Here's how the part is built. I have some questions about the finished solid (model axes, mm). Face numbers are marked on the shaded views. A direction names the side the tool comes from. Give positions to 0.01 mm unless a question says otherwise; leave off trailing zeros. Write each loop counter-clockwise with the first axis right and the second up, starting at its lowest first coordinate (ties: lowest second). Pieces come first, ordered by that corner, then holes. Notation, with made-up numbers: (37, 69.5) - (46, 69.5) arc R35 cw to (46, 108.5) - close; hole circle Ø8 at (62, -12). An arc over 180 degrees is marked (long way). One line per item, written item: value. Start each with the question number.
1) Please list where these lines run through material, in increasing order: L1, parallel to X at y = -164, z = 3.75; L2, parallel to Z at x = 255.5, y = -168.75; L3, parallel to Y at x = 255, z = 1.5. Write a range as [from, to].
2) Imagine slicing it at C-C on x = 252.75. Write out the boundary of the cut face in (y, z).
3) Imagine slicing it at B-B on x = 257.25. Write out the boundary of the cut face in (y, z), plus the area to 3 significant figures.
4) Imagine slicing it at A-A on z = 0. Write out the boundary of the cut face in (x, y), plus the area to 3 significant figures.
5) I'm going to push flat-ended pins straight in: P1, Ø5, axis at x = 256.5, y = -165.5, coming from the +Z side; P2, Ø8, axis at x = 251, z = -0.5, coming from the +Y side; P3, Ø2, axis at x = 256.5, z = -4.5, coming from the -Y side. Where does each tip first touch, or does it pass through?
6) On a 3-axis mill with a long thin cutter (end or side, diameter ignored), from which of +Z, -Z, +X, -X, +Y, -Y can I reach the whole of each face in a straight line? I mean the marked faces 1 and 2. Say none if no direction works.
from build123d import *

# Parameters (mm, degrees)
CHAMFER_1_SIZE = 1


with BuildPart() as part:
    # 草图1 → 旋转1 (revolve)
    with BuildSketch(Plane.XY, mode=Mode.PRIVATE) as revolve_1_sk:
        Polygon((236.937142185, -170.509032878), (236.937142185, -164.259032878), (256.937142185, -164.259032878), (256.937142185, -160.509032878), (261.937142185, -160.509032878), (261.937142185, -170.509032878), align=None)
    revolve(revolve_1_sk.sketch.rotate(Axis((232.937142185, -170.509032878, 0), (1, 0, 0)), 90), axis=Axis((232.937142185, -170.509032878, 0), (1, 0, 0)))

    # 倒角1
    chamfer_1_edges = [part.edges().sort_by_distance(p)[0] for p in [
        (261.937142185, -170.509032878, -10),
        (256.937142185, -170.509032878, -10),
        (236.937142185, -170.509032878, -6.25),
    ]]
    chamfer(chamfer_1_edges, length=CHAMFER_1_SIZE)


solid = part.part
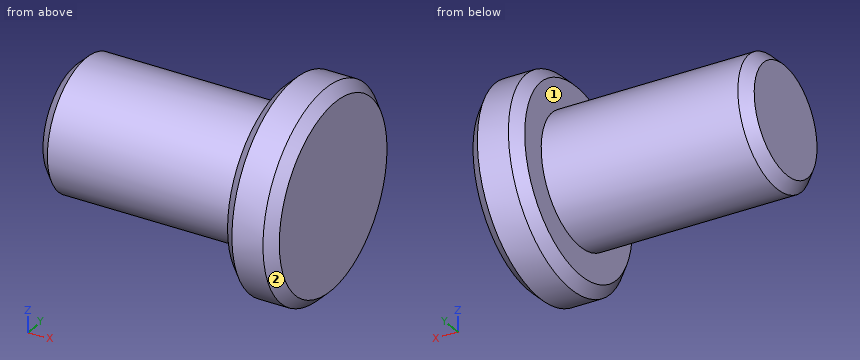
Numbers:
1. L1: [256.94, 261.94]
1. L2: [-6, 6]
1. L3: [-176.58, -164.44]
2. outline: circle Ø12.5 at (-170.51, 0)
3. outline: circle Ø18.63 at (-170.51, 0)
3. area: 272 mm^2
4. outline: (236.94, -175.76) - (237.94, -176.76) - (256.94, -176.76) - (256.94, -179.51) - (257.94, -180.51) - (260.94, -180.51) - (261.94, -179.51) - (261.94, -161.51) - (260.94, -160.51) - (257.94, -160.51) - (256.94, -161.51) - (256.94, -164.26) - (237.94, -164.26) - (236.94, -165.26) - close
4. area: 347 mm^2
5. P1: z = 9.55
5. P2: y = -164.26
5. P3: y = -179.06
6. face 1: -X
6. face 2: +X
